Read the model definition and answer for the solid it produces. Units are mm, in the model's axes. A direction names the side the tool comes from. Coordinates: 2 decimals unless noted, no trailing zeros. Loops run counter-clockwise (first coordinate to the right, second up) from the corner with the lowest first, then second, coordinate; pieces in that order, holes last. Notation, with made-up numbers: (-18.5, 22) -> (-2.5, 22) arc R14 cw to (-2.5, 34) -> close; hole circle Ø7 at (-8.5, -18.5). An arc over 180 degrees is marked (long way). Answer in a Markdown table with one row per item.
```python
from build123d import *

# Parameters (mm, degrees)
SKETCH1_R           = 1.5
SKETCH1_R_2         = 2
BOSS_EXTRUDE1_DEPTH = 1.5


with BuildPart() as part:
    # Sketch1 → Boss-Extrude1 (new, symmetric)
    with BuildSketch(Plane.XY):
        with BuildLine():
            Line((-3, 0), (-3, -6))
            ThreePointArc((-3, -6), (-2.258342613, -7.231537749), (-2, -8.645751311))
            Line((-2, -8.645751311), (-2, -25.535898385))
            ThreePointArc((-2, -25.535898385), (-2.535898385, -27.535898385), (-4, -29))
            Line((-4, -29), (-4, -35))
            ThreePointArc((-4, -35), (0, -39), (4, -35))
            Line((4, -35), (4, -29))
            ThreePointArc((4, -29), (2.535898385, -27.535898385), (2, -25.535898385))
            Line((2, -25.535898385), (2, -8.645751311))
            ThreePointArc((2, -8.645751311), (2.258342613, -7.231537749), (3, -6))
            Line((3, -6), (3, 0))
            ThreePointArc((3, 0), (0, 3), (-3, 0))
        make_face()
        Circle(SKETCH1_R, mode=Mode.SUBTRACT)
        with Locations((0, -35)):
            Circle(SKETCH1_R_2, mode=Mode.SUBTRACT)
    extrude(amount=BOSS_EXTRUDE1_DEPTH, both=True)


solid = part.part
```
1. Given pin 1 Ø0.9 at (y, z) = (-3, 0.5) entering from -X; pin 2 Ø0.9 at (y, z) = (-14, -0.5) entering from -X; pin 3 Ø1.5 at (y, z) = (-14.5, 0.5) entering from +X, each flat-ended and moving along its own axis, determine where each tip first touches the part or whether it passes through.
A:
| item | result |
|---|---|
| pin 1 | stops at x = -3 |
| pin 2 | stops at x = -2 |
| pin 3 | stops at x = 2 |
2. A cutting plane is placed at A-A on x = 0. Give the vertices of the cut face in (y, z), and give its area (3 significant figures).
A:
| item | result |
|---|---|
| outline | (-39, -1.5) -> (-37, -1.5) -> (-37, 1.5) -> (-39, 1.5) -> close; (-33, -1.5) -> (-1.5, -1.5) -> (-1.5, 1.5) -> (-33, 1.5) -> close; (1.5, -1.5) -> (3, -1.5) -> (3, 1.5) -> (1.5, 1.5) -> close |
| area | 105 mm2 |
3. A cutting plane is placed at D-D on y = -20.5. Give the vertices of the cut face in (x, z), and give its area (3 significant figures).
A:
| item | result |
|---|---|
| outline | (-2, -1.5) -> (2, -1.5) -> (2, 1.5) -> (-2, 1.5) -> close |
| area | 12.0 mm2 |
4. A cutting plane is placed at B-B on z = -0.25. Give the vertices of the cut face in (x, y), and give its area (3 significant figures).
A:
| item | result |
|---|---|
| outline | (-4, -35) arc R4 ccw to (4, -35) -> (4, -29) arc R4 cw to (2, -25.54) -> (2, -8.65) arc R4 cw to (3, -6) -> (3, 0) arc R3 ccw to (-3, 0) -> (-3, -6) arc R4 cw to (-2, -8.65) -> (-2, -25.54) arc R4 cw to (-4, -29) -> close; hole circle Ø4 at (0, -35); hole circle Ø3 at (0, 0) |
| area | 201 mm2 |
5. A cutting plane is placed at C-C on x = 2.5. Give the vertices of the cut face in (y, z).
A:
| item | result |
|---|---|
| outline | (-38.12, -1.5) -> (-27.47, -1.5) -> (-27.47, 1.5) -> (-38.12, 1.5) -> close; (-6.71, -1.5) -> (1.66, -1.5) -> (1.66, 1.5) -> (-6.71, 1.5) -> close |
6. The mould has two halves that part along X. Classify faces 4 (the cylindrical face through (-1.5, 0.07, -0.02)), 5 (the flat face through (0, -18, -1.5)), 6 (the cylindrical face through (2.25, -7.25, 0.02)), 7 (the cylindrical face through (-2.52, -27.51, 0.02)): pulls with the +X half, pulls with the -X half, needs draft (parallel to the pull), parting line crosses it, or undercut.
A:
| item | result |
|---|---|
| face 4 | undercut |
| face 5 | needs draft |
| face 6 | pulls with the +X half |
| face 7 | pulls with the -X half |
7. A tool of negligible diameter and unlimited length cuts with its end or side. For faces 1 (the flat face through (2, -17, 0)), 2 (the flat face through (-3, -3, 0)), 3 (the flat face through (3, -3, 0)), from which of +Z, -Z, +X, -X, +Y, -Y can it reach the whole face along a straight path? Write none if from no direction.
A:
| item | result |
|---|---|
| face 1 | +Z, -Z, +X |
| face 2 | +Z, -Z, -X, +Y |
| face 3 | +Z, -Z, +X, +Y |
8. Find the intervals of material crossed by probe 1 along Y at (x, z) = (0, 0.6); probe 2 along Y at (x, z) = (1.25, 1.25); probe 3 along X at (y, z) = (-14, -0.95), in increasing order.
A:
| item | result |
|---|---|
| probe 1 | y = -39 to -37, -33 to -1.5, 1.5 to 3 |
| probe 2 | y = -38.8 to -36.56, -33.44 to -0.83, 0.83 to 2.73 |
| probe 3 | x = -2 to 2 |
